```python
from build123d import *

# Parameters (mm, degrees)
BASE_BLOCK_PROFILE_W           = 70
BASE_BLOCK_PROFILE_H           = 80
BASE_BLOCK_20MM_DEPTH          = 20
H_BOSS_PROFILE_W               = 15
H_BOSS_PROFILE_H               = 25
H_BOSS_10MM_DEPTH              = 10
REAR_BOSS_PROFILE_W            = 70
REAR_BOSS_PROFILE_H            = 50
REAR_BOSS_25MM_DEPTH           = 25
REAR_BOSS_EXTENSION_PROFILE_W  = 70
REAR_BOSS_EXTENSION_PROFILE_H  = 50
REAR_BOSS_EXTENSION_25MM_DEPTH = 25
THROUGH_SLOT_8X30_DEPTH        = 100
LOWER_NOTCH_CUT_DEPTH          = 100


with BuildPart() as part:
    # Base Block Profile → Base Block 20mm (new body)
    with BuildSketch(Plane.XY):
        with Locations((35, 40)):
            Rectangle(BASE_BLOCK_PROFILE_W, BASE_BLOCK_PROFILE_H)
    extrude(amount=BASE_BLOCK_20MM_DEPTH)

    # H Boss Profile → H Boss 10mm (add)
    with BuildSketch(Plane.XY.offset(20)):
        with Locations((7.5, 67.5)):
            Rectangle(H_BOSS_PROFILE_W, H_BOSS_PROFILE_H)
        with Locations((62.5, 67.5)):
            Rectangle(H_BOSS_PROFILE_W, H_BOSS_PROFILE_H)
        with Locations((7.5, 12.5)):
            Rectangle(H_BOSS_PROFILE_W, H_BOSS_PROFILE_H)
        with Locations((62.5, 12.5)):
            Rectangle(H_BOSS_PROFILE_W, H_BOSS_PROFILE_H)
    extrude(amount=H_BOSS_10MM_DEPTH)

    # Rear Boss Profile → Rear Boss 25mm (add)
    with BuildSketch(Plane(origin=(0, 80, 0), x_dir=(1, 0, 0), z_dir=(0, 1, 0))):
        with Locations((35, 25)):
            Rectangle(REAR_BOSS_PROFILE_W, REAR_BOSS_PROFILE_H)
    extrude(amount=-REAR_BOSS_25MM_DEPTH)

    # Rear Boss Extension Profile → Rear Boss Extension 25mm (add)
    with BuildSketch(Plane.XZ):
        with Locations((35, -25)):
            Rectangle(REAR_BOSS_EXTENSION_PROFILE_W, REAR_BOSS_EXTENSION_PROFILE_H)
    extrude(amount=-REAR_BOSS_EXTENSION_25MM_DEPTH)

    # Slot 8x30 Profile → Through Slot 8x30 (cut)
    with BuildSketch(Plane.XZ):
        with BuildLine():
            Line((20, -20), (50, -20))
            ThreePointArc((50, -20), (58, -28), (50, -36))
            Line((50, -36), (20, -36))
            ThreePointArc((20, -36), (12, -28), (20, -20))
        make_face()
    extrude(amount=-THROUGH_SLOT_8X30_DEPTH, mode=Mode.SUBTRACT)

    # Lower Notch Profile → Lower Notch Cut (cut)
    with BuildSketch(Plane.XZ):
        with BuildLine():
            Line((0, -50), (0, -30))
            ThreePointArc((0, -30), (5.857864376, -44.142135624), (20, -50))
            Line((20, -50), (0, -50))
        make_face()
        with BuildLine():
            Line((70, -50), (70, -30))
            ThreePointArc((70, -30), (64.142135624, -44.142135624), (50, -50))
            Line((50, -50), (70, -50))
        make_face()
    extrude(amount=-LOWER_NOTCH_CUT_DEPTH, mode=Mode.SUBTRACT)


solid = part.part
```
Read the model definition and answer for the solid it produces. Units are mm, in the model's axes. A direction names the side the tool comes from. Round coordinates to 2 decimals unless told otherwise and drop trailing zeros. Write each loop counter-clockwise with the first axis right and the second up, starting at its lowest first coordinate (ties: lowest second). Pieces come first, ordered by that corner, then holes. Notation, with made-up numbers: M -21.5,83.5 L -3.5,83.5 A17 cw -3.5,91.5 Z; hole C -23,35 d5. An arc over 180 degrees is marked long. One line per item, written item: value.
Q1. Find section A-A on z = -16. Write down the section's boundary in (x, y), plus the area to 3 significant figures.
Data:
outline: M 0,0 L 70,0 L 70,25 L 0,25 Z; M 0,55 L 70,55 L 70,80 L 0,80 Z
area: 3,500 mm2
Q2. Straight lines are drawn through the part: line 1 (Y direction, x = 9, z = -17.5); line 2 (Z direction, x = 26, y = 68); line 3 (Z direction, x = 41.5, y = 29). For each, find the intervals that lie inside material, in ascending order. Write a range as [from, to].
Data:
line 1: [0, 25], [55, 80]
line 2: [-50, -36], [-20, 20]
line 3: [0, 20]
Q3. Flat-ended cylindrical pins translate along their axes: pin 1 Ø25 at (x, z) = (22, -20.5) entering from +Y; pin 2 Ø5 at (x, y) = (36.5, 33.5) entering from +Z; pin 3 Ø9 at (x, y) = (38, 45.5) entering from -Z. Find the tip coordinate at first contact, or state that the pin passes through.
Data:
pin 1: y = 80
pin 2: z = 20
pin 3: z = 0
Q4. For a pull along X with two mould halves and no side action, classify faces 1 (the flat face through (35, 40, 0)), 2 (the cylindrical face through (12, 67, -28)), 3 (the cylindrical face through (5.703, 67.325, -43.986)) as +X half, -X half, draft (parallel to the pull), parting line (faces both ways), or undercut.
Data:
face 1: draft
face 2: undercut
face 3: -X half
Q5. Which of the six approach directions +Z, -Z, +X, -X, +Y, -Y give full straight-line access (tool end or side, diameter ignored) to faces 4 (the flat face through (35, 12, -36)), 5 (the flat face through (15, 67, 25)), 6 (the flat face through (7, 55, 25)), 7 (the flat face through (34.5, 55, -19.8))?
Data:
face 4: +Y, -Y
face 5: +Z, +Y, -Y
face 6: +Z, +X, -X
face 7: -Z, +X, -X
Q6. Find section C-C on y = 13. Write down the section's boundary in (x, z).
Data:
outline: M 0,-30 A20 ccw 20,-50 L 50,-50 A20 ccw 70,-30 L 70,30 L 55,30 L 55,20 L 15,20 L 15,30 L 0,30 Z; hole M 20,-36 L 50,-36 A8 ccw 50,-20 L 20,-20 A8 ccw Z
Q7. Find section B-B on x = 35. Write down the section's boundary in (y, z), plus the area to 3 significant figures.
Data:
outline: M 0,-50 L 25,-50 L 25,-36 L 0,-36 Z; M 0,-20 L 25,-20 L 25,0 L 55,0 L 55,-20 L 80,-20 L 80,20 L 0,20 Z; M 55,-50 L 80,-50 L 80,-36 L 55,-36 Z
area: 3,300 mm2
Q8. Find section D-D on z = -28. Write down the section's boundary in (x, y).
Data:
outline: M 0,0 L 12,0 L 12,25 L 0,25 Z; M 0,55 L 12,55 L 12,80 L 0,80 Z; M 58,0 L 70,0 L 70,25 L 58,25 Z; M 58,55 L 70,55 L 70,80 L 58,80 Z
